```python
from build123d import *

# Parameters (mm, degrees)
BASE_PLATE_SKETCH_W  = 6
BASE_PLATE_SKETCH_H  = 6
BASE_PLATE_DEPTH     = 1
UPPER_PAD_SKETCH_W   = 6
UPPER_PAD_SKETCH_H   = 1
UPPER_PAD_DEPTH      = 1.5
LOWER_PAD_SKETCH_W   = 6
LOWER_PAD_SKETCH_H   = 1
LOWER_PAD_DEPTH      = 1.5
NOTCH_CUTS_DEPTH     = 1.5
STEM_SKETCH_W        = 3
STEM_SKETCH_H        = 1
STEM_1X3_DEPTH       = 4
STEM_FILLET_R0_5_A_R = 0.5
STEM_FILLET_R0_5_B_R = 0.5
LUG_PLATE_SKETCH_R   = 0.75
LUG_PLATE_DEPTH      = 1


with BuildPart() as part:
    # Base Plate Sketch → Base Plate (new body)
    with BuildSketch(Plane.XY):
        Rectangle(BASE_PLATE_SKETCH_W, BASE_PLATE_SKETCH_H)
    extrude(amount=-BASE_PLATE_DEPTH)

    # Upper Pad Sketch → Upper Pad (add)
    with BuildSketch(Plane(origin=(0, 3, 0), x_dir=(1, 0, 0), z_dir=(0, 1, 0))):
        with Locations((0, 0.5)):
            Rectangle(UPPER_PAD_SKETCH_W, UPPER_PAD_SKETCH_H)
    extrude(amount=UPPER_PAD_DEPTH)

    # Lower Pad Sketch → Lower Pad (add)
    with BuildSketch(Plane.XZ.offset(3)):
        with Locations((0, -0.5)):
            Rectangle(LOWER_PAD_SKETCH_W, LOWER_PAD_SKETCH_H)
    extrude(amount=LOWER_PAD_DEPTH)

    # Notch Cut Sketch → Notch Cuts (cut)
    with BuildSketch(Plane.XY):
        with BuildLine():
            Line((-1.5, 3.5), (-3, 3.5))
            Line((-3, 3.5), (-3, 1.5))
            Line((-3, 1.5), (-1.5, 1.5))
            ThreePointArc((-1.5, 1.5), (-0.5, 2.5), (-1.5, 3.5))
        make_face()
        with BuildLine():
            Line((1.5, 3.5), (3, 3.5))
            Line((3, 3.5), (3, 1.5))
            Line((3, 1.5), (1.5, 1.5))
            ThreePointArc((1.5, 1.5), (0.5, 2.5), (1.5, 3.5))
        make_face()
        with BuildLine():
            Line((3, -1.5), (3, -3.5))
            Line((3, -3.5), (1.5, -3.5))
            ThreePointArc((1.5, -3.5), (0.5, -2.5), (1.5, -1.5))
            Line((1.5, -1.5), (3, -1.5))
        make_face()
        with BuildLine():
            Line((-1.5, -1.5), (-3, -1.5))
            Line((-3, -1.5), (-3, -3.5))
            Line((-3, -3.5), (-1.5, -3.5))
            ThreePointArc((-1.5, -3.5), (-0.5, -2.5), (-1.5, -1.5))
        make_face()
    extrude(amount=-NOTCH_CUTS_DEPTH, mode=Mode.SUBTRACT)

    # Stem Sketch → Stem 1x3 (add)
    with BuildSketch(Plane.XY):
        with Locations((0, -0.5)):
            Rectangle(STEM_SKETCH_W, STEM_SKETCH_H)
    extrude(amount=STEM_1X3_DEPTH)

    # Stem Fillet R0.5 A
    stem_fillet_r0_5_a_edges = [part.edges().sort_by_distance(p)[0] for p in [
        (1.5, -0.5, 0),
    ]]
    fillet(stem_fillet_r0_5_a_edges, radius=STEM_FILLET_R0_5_A_R)

    # Stem Fillet R0.5 B
    stem_fillet_r0_5_b_edges = [part.edges().sort_by_distance(p)[0] for p in [
        (-1.5, -0.5, 0),
    ]]
    fillet(stem_fillet_r0_5_b_edges, radius=STEM_FILLET_R0_5_B_R)

    # Lug Plate Sketch → Lug Plate (add)
    with BuildSketch(Plane.XY.offset(4)):
        with BuildLine():
            Line((1.5, 3), (1.5, -3))
            ThreePointArc((1.5, -3), (0, -4.5), (-1.5, -3))
            Line((-1.5, -3), (-1.5, 3))
            ThreePointArc((-1.5, 3), (0, 4.5), (1.5, 3))
        make_face()
        with Locations((0, 3)):
            Circle(LUG_PLATE_SKETCH_R, mode=Mode.SUBTRACT)
        with Locations((0, -3)):
            Circle(LUG_PLATE_SKETCH_R, mode=Mode.SUBTRACT)
    extrude(amount=LUG_PLATE_DEPTH)


solid = part.part
```
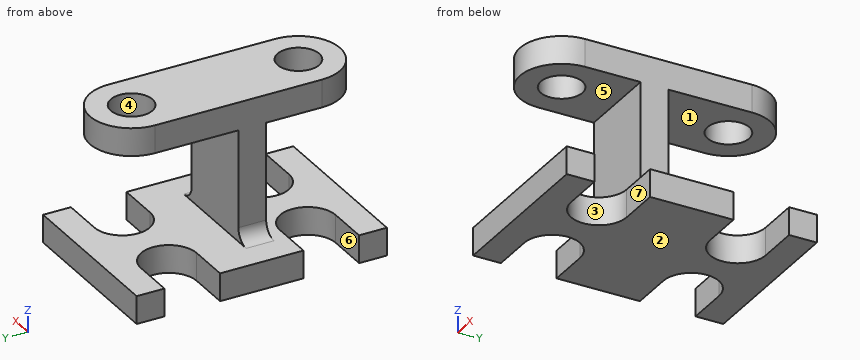
Part model, mm, in its own coordinate system. Face numbers are marked on the shaded views. A direction names the side the tool comes from. Round coordinates to 2 decimals unless told otherwise and drop trailing zeros. Order: outer loops, then holes, each group sorted by start corner. A loop starts at its lowest first (then second) coordinate and runs counter-clockwise, first axis right, second up. Notation, with made-up numbers: M 8,48.25 L 25,48.25 A28 cw 25,82.25 Z; hole C 83,65.25 d8. An arc over 180 degrees is marked long. Put each result on its own line as item: value. Start each with the question number.
1. Drill centre lines: probe 1 along Y at (x, z) = (0, 4.5); probe 2 along Z at (x, y) = (-1.35, 0.5); probe 3 along Z at (x, y) = (-1.8, 0.25). Where is each one in solid material? Low to high. Write a range as [from, to].
2. Tool access for the marked faces 4, 5, 6 and 7: list every direction of +Z, -Z, +X, -X, +Y, -Y with a clear straight run to the whole face (end or side of a thin tool).
3. Slice it at A-A on y = 1.25. List the corners of the cut face in (x, z).
4. Slice it at B-B on x = 0. List the corners of the cut face in (y, z).
5. Two-plate mould, pull along Z, no slides. Class the marked faces 1, 2 and 3: +Z half, -Z half, draft (parallel to the pull), parting line (faces both ways), or undercut.
6. Slice it at C-C on z = 4.3. List the corners of the cut face in (x, y).
7. Drop flat-ended pins along their axis: pin 1 (1 mm diameter, centred on x = 0.5, y = -3.5, fed in from +Z); pin 2 (1.2 mm diameter, centred on x = 0.5, z = 2, fed in from -Y); pin 3 (3.5 mm diameter, centred on y = 1, z = 3, fed in from +X). Give the stop position or say it passes through.
8. Slice it at D-D on y = 2.5. List the corners of the cut face in (x, z), then the cut area to 3 significant figures.
Findings:
1. probe 1: [-4.5, -3.75], [-2.25, 2.25], [3.75, 4.5]
1. probe 2: [-1, 0], [4, 5]
1. probe 3: [-1, 0]
2. face 4: +Z
2. face 5: +X, -X, -Y
2. face 6: +Z, -Z, -X
2. face 7: +Z, -Z, +X
3. outline: M -3,-1 L 3,-1 L 3,0 L -3,0 Z; M -1.5,4 L 1.5,4 L 1.5,5 L -1.5,5 Z
4. outline: M -4.5,-1 L 4.5,-1 L 4.5,0 L 0,0 L 0,4 L 2.25,4 L 2.25,5 L -2.25,5 L -2.25,4 L -1,4 L -1,0 L -4.5,0 Z; M -4.5,4 L -3.75,4 L -3.75,5 L -4.5,5 Z; M 3.75,4 L 4.5,4 L 4.5,5 L 3.75,5 Z
5. face 1: undercut
5. face 2: -Z half
5. face 3: draft
6. outline: M -1.5,-3 A1.5 ccw 1.5,-3 L 1.5,3 A1.5 ccw -1.5,3 Z; hole C 0,-3 d1.5; hole C 0,3 d1.5
7. pin 1: z = 5
7. pin 2: y = -1
7. pin 3: x = 1.5
8. outline: M -1.5,4 L -0.56,4 L -0.56,5 L -1.5,5 Z; M -0.5,-1 L 0.5,-1 L 0.5,0 L -0.5,0 Z; M 0.56,4 L 1.5,4 L 1.5,5 L 0.56,5 Z
8. area: 2.88 mm2
